Source: three-view drawing plus pictorial views. Frame: mm from the lowest corner of the part. A direction names the side the tool comes from. Give positions to 0.01 mm unless a question says otherwise; leave off trailing zeros. Order: outer loops, then holes, each group sorted by start corner. A loop starts at its lowest first (then second) coordinate and runs counter-clockwise, first axis right, second up. Notation, with made-up numbers: M 9,21 L 36,21 A23 cw 36,52 Z; hole C 9,-20 d2. An arc over 180 degrees is marked long. Use CSV: the item, a comma, the result in double quotes. Start each with the question number.
Item 1: Access query for the marked faces 5 and 6. Directions: +Z, -Z, +X, -X, +Y, -Y. A direction counts if a zero-diameter tool reaches every point of the face in a straight line with its end or side. Return the directions, or none.
Item 2: Section query B-B on z = 33. Return loops of the section in (x, y).
Item 3: Section query C-C on x = 109. Return loops of the section in (y, z).
Item 4: Section query A-A on y = 6.5. Return loops of the section in (x, z), and give its area (3 significant figures).
Item 5: First-contact query: pin 1 (1 mm diameter, centred on y = 6.5, z = 52.5, fed in from -X); pin 2 (4 mm diameter, centred on x = 52, y = 2.5, fed in from +Z); pin 3 (6 mm diameter, centred on y = 6.5, z = 29, fed in from +X); pin 4 (5 mm diameter, centred on x = 4, y = 4, fed in from -Z). Flat tips, straight axial feed; report the tip coordinate or a pass-through.
Item 6: Ray query, probe 1 along X at (y, z) = (7.5, 36); probe 2 along Z at (x, y) = (69.5, 1.75); probe 3 along Z at (x, y) = (108.5, 6). Return the intervals inside material, ascending. Write a range as from..to.
Item 7: Pull-direction query (Z, two-part tool) for the marked faces 1, 2, 3 and 4; classes: +Z half, -Z half, draft (parallel to the pull), parting line (faces both ways), or undercut.
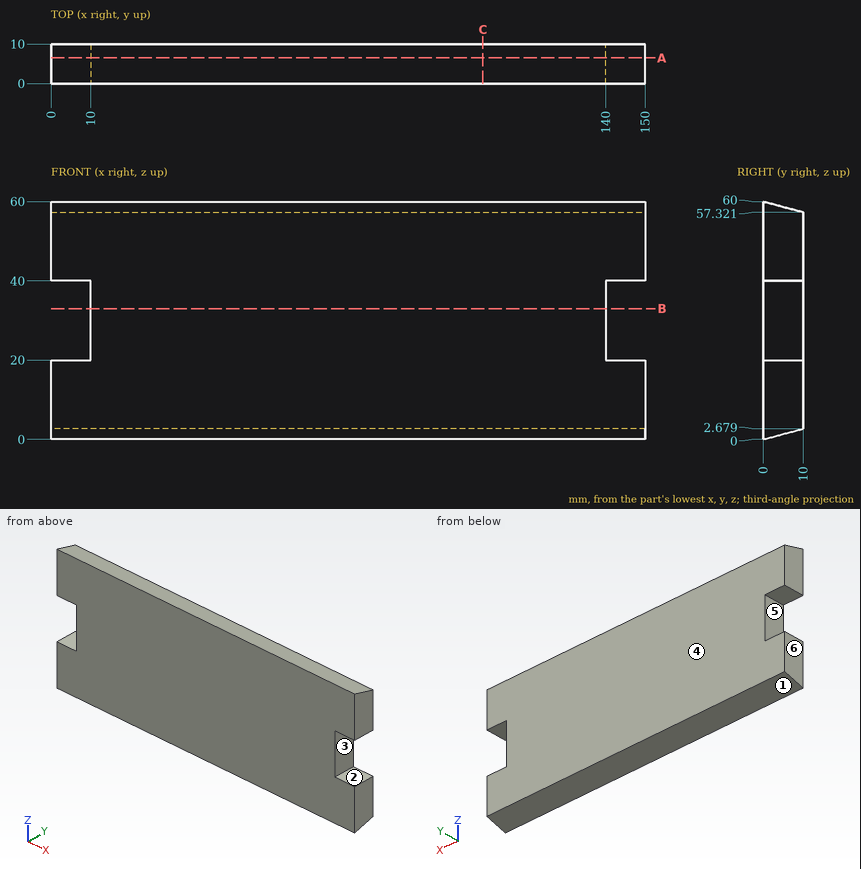
Verdict:
1,face 5,"-X, +Y, -Y"
1,face 6,"+Z, -Z, -X, +Y, -Y"
2,outline,"M 10,0 L 140,0 L 140,10 L 10,10 Z"
3,outline,"M 0,0 L 10,2.68 L 10,57.32 L 0,60 Z"
4,outline,"M 0,1.74 L 150,1.74 L 150,20 L 140,20 L 140,40 L 150,40 L 150,58.26 L 0,58.26 L 0,40 L 10,40 L 10,20 L 0,20 Z"
4,area,"8,080 mm2"
5,pin 1,"x = 0"
5,pin 2,"z = 59.87"
5,pin 3,"x = 140"
5,pin 4,"z = 0.4"
6,probe 1,"10..140"
6,probe 2,"0.47..59.53"
6,probe 3,"1.61..58.39"
7,face 1,"-Z half"
7,face 2,"undercut"
7,face 3,"undercut"
7,face 4,"draft"
